```python
from build123d import *

# Parameters (mm, degrees)
SKETCH_1_W                = 60
SKETCH_1_H                = 345
EXTRUDE_1_DEPTH           = 16
HOLE_WIZARD_1_D           = 9
HOLE_WIZARD_1_CBORE_D     = 15
HOLE_WIZARD_1_CBORE_DEPTH = 9
CHAMFER_1_SIZE            = 2
CUT_EXTRUDE_3_DEPTH       = 9
CUT_EXTRUDE_4_DEPTH       = 176.320420944
HOLE_WIZARD_M10_1_D       = 8.5
HOLE_WIZARD_M10_1_DEPTH   = 27.5
HOLE_WIZARD_M10_1_TIP     = 2.553657631
MM_1_D                    = 10
MM_1_DEPTH                = 25
MM_1_TIP                  = 3.004303095


with BuildPart() as part:
    # 草图1 → 凸台-拉伸1 (new body)
    with BuildSketch(Plane.XY):
        Rectangle(SKETCH_1_W, SKETCH_1_H)
    extrude(amount=EXTRUDE_1_DEPTH)

    # 打孔尺寸(%根据)内六角圆柱头螺钉的类型1 (through all)
    with Locations(Plane.XY.offset(16)):
        with Locations((18, 147.5), (-18, -82.5), (-18, 147.5), (18, -82.5), (-18, 32.5), (18, 32.5)):
            CounterBoreHole(HOLE_WIZARD_1_D / 2, HOLE_WIZARD_1_CBORE_D / 2, HOLE_WIZARD_1_CBORE_DEPTH)

    # 倒角1
    chamfer_1_edges = [part.edges().sort_by_distance(p)[0] for p in [
        (30, -172.5, 8),
        (-30, -172.5, 8),
        (-30, 172.5, 8),
        (30, 172.5, 8),
    ]]
    chamfer(chamfer_1_edges, length=CHAMFER_1_SIZE)

    # 草图7 → 切除-拉伸3 (cut)
    with BuildSketch(Plane.XY.offset(16)):
        with BuildLine():
            Line((-10.5, 157.5), (-10.5, 137.5))
            ThreePointArc((-10.5, 137.5), (-18, 130), (-25.5, 137.5))
            Line((-25.5, 137.5), (-25.5, 157.5))
            ThreePointArc((-25.5, 157.5), (-18, 165), (-10.5, 157.5))
        make_face()
        with BuildLine():
            Line((25.5, 157.5), (25.5, 137.5))
            ThreePointArc((25.5, 137.5), (18, 130), (10.5, 137.5))
            Line((10.5, 137.5), (10.5, 157.5))
            ThreePointArc((10.5, 157.5), (18, 165), (25.5, 157.5))
        make_face()
        with BuildLine():
            Line((-25.5, 22.5), (-25.5, 42.5))
            ThreePointArc((-25.5, 42.5), (-18, 50), (-10.5, 42.5))
            Line((-10.5, 42.5), (-10.5, 22.5))
            ThreePointArc((-10.5, 22.5), (-18, 15), (-25.5, 22.5))
        make_face()
        with BuildLine():
            Line((10.5, 22.5), (10.5, 42.5))
            ThreePointArc((10.5, 42.5), (18, 50), (25.5, 42.5))
            Line((25.5, 42.5), (25.5, 22.5))
            ThreePointArc((25.5, 22.5), (18, 15), (10.5, 22.5))
        make_face()
        with BuildLine():
            Line((-25.5, -92.5), (-25.5, -72.5))
            ThreePointArc((-25.5, -72.5), (-18, -65), (-10.5, -72.5))
            Line((-10.5, -72.5), (-10.5, -92.5))
            ThreePointArc((-10.5, -92.5), (-18, -100), (-25.5, -92.5))
        make_face()
        with BuildLine():
            Line((10.5, -92.5), (10.5, -72.5))
            ThreePointArc((10.5, -72.5), (18, -65), (25.5, -72.5))
            Line((25.5, -72.5), (25.5, -92.5))
            ThreePointArc((25.5, -92.5), (18, -100), (10.5, -92.5))
        make_face()
    extrude(amount=-CUT_EXTRUDE_3_DEPTH, mode=Mode.SUBTRACT)

    # 草图8 → 切除-拉伸4 (cut, through all)
    with BuildSketch(Plane.XY.offset(7)):
        with BuildLine():
            Line((-22.5, 137.5), (-22.5, 157.5))
            ThreePointArc((-22.5, 157.5), (-18, 162), (-13.5, 157.5))
            Line((-13.5, 157.5), (-13.5, 137.5))
            ThreePointArc((-13.5, 137.5), (-18, 133), (-22.5, 137.5))
        make_face()
        with BuildLine():
            Line((13.5, 137.5), (13.5, 157.5))
            ThreePointArc((13.5, 157.5), (18, 162), (22.5, 157.5))
            Line((22.5, 157.5), (22.5, 137.5))
            ThreePointArc((22.5, 137.5), (18, 133), (13.5, 137.5))
        make_face()
        with BuildLine():
            Line((-22.5, 22.5), (-22.5, 42.5))
            ThreePointArc((-22.5, 42.5), (-18, 47), (-13.5, 42.5))
            Line((-13.5, 42.5), (-13.5, 22.5))
            ThreePointArc((-13.5, 22.5), (-18, 18), (-22.5, 22.5))
        make_face()
        with BuildLine():
            Line((13.5, 22.5), (13.5, 42.5))
            ThreePointArc((13.5, 42.5), (18, 47), (22.5, 42.5))
            Line((22.5, 42.5), (22.5, 22.5))
            ThreePointArc((22.5, 22.5), (18, 18), (13.5, 22.5))
        make_face()
        with BuildLine():
            Line((-22.5, -92.5), (-22.5, -72.5))
            ThreePointArc((-22.5, -72.5), (-18, -68), (-13.5, -72.5))
            Line((-13.5, -72.5), (-13.5, -92.5))
            ThreePointArc((-13.5, -92.5), (-18, -97), (-22.5, -92.5))
        make_face()
        with BuildLine():
            Line((13.5, -92.5), (13.5, -72.5))
            ThreePointArc((13.5, -72.5), (18, -68), (22.5, -72.5))
            Line((22.5, -72.5), (22.5, -92.5))
            ThreePointArc((22.5, -92.5), (18, -97), (13.5, -92.5))
        make_face()
    extrude(amount=-CUT_EXTRUDE_4_DEPTH, mode=Mode.SUBTRACT)

    # M10 螺纹孔1
    with Locations(Plane.XY.offset(16)):
        with Locations((-18, 107.5), (18, 107.5), (-18, -157.5), (18, -157.5)):
            Hole(HOLE_WIZARD_M10_1_D / 2, depth=HOLE_WIZARD_M10_1_DEPTH)
            with Locations((0, 0, -(HOLE_WIZARD_M10_1_DEPTH + HOLE_WIZARD_M10_1_TIP / 2))):  # 118° drill point
                Cone(0, HOLE_WIZARD_M10_1_D / 2, HOLE_WIZARD_M10_1_TIP, mode=Mode.SUBTRACT)

    # 大小mm 暗销孔1
    with Locations(Plane.XY.offset(16)):
        with Locations((0, -57.5), (0, 122.5)):
            Hole(MM_1_D / 2, depth=MM_1_DEPTH)
            with Locations((0, 0, -(MM_1_DEPTH + MM_1_TIP / 2))):  # 118° drill point
                Cone(0, MM_1_D / 2, MM_1_TIP, mode=Mode.SUBTRACT)


solid = part.part
```
The listing builds one solid part. Answer for the finished solid, in the listing's coordinates (mm). A direction names the side the tool comes from. Give positions to 0.01 mm unless a question says otherwise; leave off trailing zeros. Order: outer loops, then holes, each group sorted by start corner. A loop starts at its lowest first (then second) coordinate and runs counter-clockwise, first axis right, second up.
Item 1: Given pin 1 Ø1 at (x, y) = (-13.5, -93) entering from +Z; pin 2 Ø1 at (x, y) = (-20.5, 39) entering from -Z, each flat-ended and moving along its own axis, determine where each tip first touches the part or whether it passes through.
From the geometry:
pin 1: stops at z = 7
pin 2: passes through
Item 2: Find the intervals of material crossed by probe 1 along X at (y, z) = (155.5, 14); probe 2 along X at (y, z) = (30, 5.5); probe 3 along Y at (x, z) = (0, 9.75), in increasing order.
From the geometry:
probe 1: x = -30 to -25.5, -10.5 to 10.5, 25.5 to 30
probe 2: x = -30 to -22.5, -13.5 to 13.5, 22.5 to 30
probe 3: y = -172.5 to -62.5, -52.5 to 117.5, 127.5 to 172.5
Item 3: The part is cut by section D-D, the plane x = -18. Count the separate pieces of the cut face and the enclosed holes in it, and give its area (3 significant figures).
From the geometry:
separate pieces: 6
enclosed holes: 0
area: 3,690 mm2
Item 4: For a pull along X with two mould halves and no side action, classify faces 4 (the face through (13.5, 32, 4)), 5 (the face through (0, 2, 0)) as pulls with the +X half, pulls with the -X half, needs draft (parallel to the pull), parting line crosses it, or undercut.
From the geometry:
face 4: undercut
face 5: needs draft
Item 5: The part is cut by section A-A, the plane x = 0. Give the vertices of the cut face in (y, z), and give its area (3 significant figures).
From the geometry:
outline: (-172.5, 0) - (-62.5, 0) - (-62.5, 16) - (-172.5, 16) - close; (-52.5, 0) - (117.5, 0) - (117.5, 16) - (-52.5, 16) - close; (127.5, 0) - (172.5, 0) - (172.5, 16) - (127.5, 16) - close
area: 5,200 mm2
Item 6: The part is cut by section B-B, the plane y = 107.5. Give the vertices of the cut face in (x, z), and give its area (3 significant figures).
From the geometry:
outline: (-30, 0) - (-22.25, 0) - (-22.25, 16) - (-30, 16) - close; (-13.75, 0) - (13.75, 0) - (13.75, 16) - (-13.75, 16) - close; (22.25, 0) - (30, 0) - (30, 16) - (22.25, 16) - close
area: 688 mm2
Item 7: Which of the six approach directions +Z, -Z, +X, -X, +Y, -Y give full straight-line access (tool end or side, diameter ignored) to faces 1 (the face through (-18, 133, 4)), 2 (the face through (0, 172.5, 8)), 3 (the face through (-18, 50, 12))?
From the geometry:
face 1: +Z, -Z
face 2: +Z, -Z, +X, -X, +Y
face 3: +Z
Item 8: The part is cut by section C-C, the plane y = -88. Give the vertices of the cut face in (x, z).
From the geometry:
outline: (-30, 0) - (-22.5, 0) - (-22.5, 7) - (-25.5, 7) - (-25.5, 16) - (-30, 16) - close; (-13.5, 0) - (13.5, 0) - (13.5, 7) - (10.5, 7) - (10.5, 16) - (-10.5, 16) - (-10.5, 7) - (-13.5, 7) - close; (22.5, 0) - (30, 0) - (30, 16) - (25.5, 16) - (25.5, 7) - (22.5, 7) - close
